from build123d import *

# Parameters (mm, degrees)
SKETCH1_R           = 4
BOSS_EXTRUDE1_DEPTH = 5
SKETCH2_R           = 2.5
BOSS_EXTRUDE2_DEPTH = 25
SKETCH3_R           = 0.75


with BuildPart() as part:
    # Sketch1 → Boss-Extrude1 (new body)
    with BuildSketch(Plane.XY):
        Circle(SKETCH1_R)
    extrude(amount=BOSS_EXTRUDE1_DEPTH)

    # Sketch2 → Boss-Extrude2 (add)
    with BuildSketch(Plane.XY.offset(5)):
        Circle(SKETCH2_R)
    extrude(amount=BOSS_EXTRUDE2_DEPTH)

    # Sweep1: sweep along a path in Sketch4
    with BuildLine(Plane(origin=(0, 0, 0), x_dir=(0, 0, -1), z_dir=(1, 0, 0))) as sweep1_path:
        Line((-2.5, 0), (-2.5, -4.330127019))
        ThreePointArc((-2.5, -4.330127019), (-1.25, -6.495190528), (1.25, -6.495190528))
        ThreePointArc((1.25, -6.495190528), (5, 0), (1.25, 6.495190528))
        ThreePointArc((1.25, 6.495190528), (-1.25, 6.495190528), (-2.5, 4.330127019))
        Line((-2.5, 4.330127019), (-2.5, 0))
    # Sketch3 → Sweep1 (sweep)
    with BuildSketch(Plane(origin=(0, 0, 0), x_dir=(1, 0, 0), z_dir=(0, 1, 0))):
        with Locations((0, -2.5)):
            Circle(SKETCH3_R)
    sweep(path=sweep1_path.line)


solid = part.part
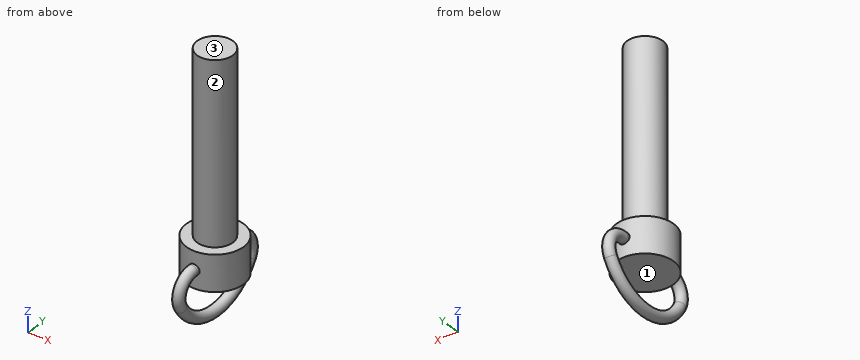
Part model, mm, in its own coordinate system. Face numbers are marked on the shaded views. Coordinates: 2 decimals unless noted, no trailing zeros. Loops run counter-clockwise (first coordinate to the right, second up) from the corner with the lowest first, then second, coordinate; pieces in that order, holes last. Notation, with made-up numbers: (17.5, 55.25) -> (72.5, 55.25) arc R20 cw to (72.5, 87.25) -> close; hole circle Ø4 at (88, 15). An arc over 180 degrees is marked (long way). Use a Markdown table: item, result. Add a question column.
Item 1: Probe probe 1 along Z at (x, y) = (-3, -1.75); probe 2 along Y at (x, z) = (0, 12); probe 3 along Z at (x, y) = (-1.5, 0). List the from-to ranges inside material, lowest first.
Item 2: Band-saw the part on C-C on z = 15. Write the cut outline in (x, y), plus the area to 3 significant figures.
Item 3: Band-saw the part on A-A on y = 0. Write the cut outline in (x, z).
Item 4: Band-saw the part on D-D on x = 1.75. Write the cut outline in (y, z).
Item 5: Pull direction Z, two halves, no side cores. Call the marked faces 1, 2 and 3: +Z half, -Z half, draft (parallel to the pull), parting line (faces both ways), or undercut.
Item 6: Flat gauge pins, fed straight in: P1, Ø4, axis at x = 2, y = -5.5, coming from the +Z side; P2, Ø3, axis at y = -1, z = 10, coming from the +X side; P3, Ø1, axis at x = 1, z = 26, coming from the +Y side. Where does each tip first touch, or does it go through?
Item 7: Band-saw the part on B-B on x = 0. Write the cut outline in (y, z) (3 decimals).
Geometry says:
| question | item | result |
|---|---|---|
| 1 | probe 1 | 0 to 5 |
| 1 | probe 2 | -2.5 to 2.5 |
| 1 | probe 3 | 0 to 30 |
| 2 | outline | circle Ø5 at (0, 0) |
| 2 | area | 19.6 mm² |
| 3 | outline | (-4, 0) -> (4, 0) -> (4, 5) -> (2.5, 5) -> (2.5, 30) -> (-2.5, 30) -> (-2.5, 5) -> (-4, 5) -> close; circle Ø1.5 at (0, -5) |
| 4 | outline | (-3.6, 0) -> (3.6, 0) -> (3.6, 5) -> (1.79, 5) -> (1.79, 30) -> (-1.79, 30) -> (-1.79, 5) -> (-3.6, 5) -> close |
| 5 | face 1 | undercut |
| 5 | face 2 | draft |
| 5 | face 3 | +Z half |
| 6 | P1 | z = 5 |
| 6 | P2 | x = 2.5 |
| 6 | P3 | y = 2.45 |
| 7 | outline | (-7.145, -1.625) arc R8.25 ccw to (7.145, -1.625) arc R3.25 ccw to (4.33, 3.25) -> (4, 3.25) -> (4, 5) -> (2.5, 5) -> (2.5, 30) -> (-2.5, 30) -> (-2.5, 5) -> (-4, 5) -> (-4, 3.25) -> (-4.33, 3.25) arc R3.25 ccw to start; hole (-5.846, -0.875) arc R6.75 ccw to (5.846, -0.875) arc R1.75 ccw to (4.33, 1.75) -> (4, 1.75) -> (4, 0) -> (-4, 0) -> (-4, 1.75) -> (-4.33, 1.75) arc R1.75 ccw to start |
